from build123d import *

# Parameters (mm, degrees)
SKETCH1_R  = 1.25
BODY_DEPTH = 1.5


with BuildPart() as part:
    # Sketch1 → Body (new body)
    with BuildSketch(Plane.XY):
        with BuildLine():
            Line((6.047730211, -14.600512296), (7.232716872, -17.461323164))
            ThreePointArc((7.232716872, -17.461323164), (0, 18.9), (-7.232716872, -17.461323164))
            Line((-7.232716872, -17.461323164), (-6.047730211, -14.600512296))
            ThreePointArc((-6.047730211, -14.600512296), (-6.904744304, -11.609176709), (-10.012271945, -11.769905381))
            ThreePointArc((-10.012271945, -11.769905381), (-11.097089224, -12.142747822), (-12.128155002, -11.64001193))
            ThreePointArc((-12.128155002, -11.64001193), (0, 15.3), (12.128155002, -11.64001193))
            ThreePointArc((12.128155002, -11.64001193), (11.097089224, -12.142747822), (10.012271945, -11.769905381))
            ThreePointArc((10.012271945, -11.769905381), (6.904744304, -11.609176709), (6.047730211, -14.600512296))
        make_face()
        with Locations(Location((8.357429042, -13.643803715, 0), (0, 0, 180))):
            Circle(SKETCH1_R, mode=Mode.SUBTRACT)
        with Locations((-8.357429042, -13.643803715)):
            Circle(SKETCH1_R, mode=Mode.SUBTRACT)
    extrude(amount=-BODY_DEPTH)


solid = part.part
Model file for the job. Use its own axes, mm. A direction names the side the tool comes from. Round coordinates to 2 decimals unless told otherwise and drop trailing zeros. Loops run counter-clockwise (first coordinate to the right, second up) from the corner with the lowest first, then second, coordinate; pieces in that order, holes last. Notation, with made-up numbers: (-23, 24.5) - (-1, 24.5) arc R19 ccw to (-1, 38.5) - close; hole circle Ø4 at (29.5, 5.25). An arc over 180 degrees is marked (long way). Write each question's results on one line, items separated by ' | '.
(1) 3-axis set-ups, long thin cutter, end or side, ignore diameter. For faces 1 (the flat face through (0, 16, -1.5)), 2 (the cylindrical face through (-11.081, -12.144, -0.74)), 3 (the flat face through (6.63, -16.01, -0.74)): which of +Z, -Z, +X, -X, +Y, -Y reach the whole face in a straight line?
Answer below:
face 1: -Z, +X, -X, +Y, -Y | face 2: +Z, -Z | face 3: +Z, -Z, -Y
(2) Saw through at B-B, the plane x = 11. List the corners of the cut face in (y, z).
Answer below:
outline: (-15.37, -1.5) - (-12.15, -1.5) - (-12.15, 0) - (-15.37, 0) - close; (10.99, -1.5) - (15.37, -1.5) - (15.37, 0) - (10.99, 0) - close
(3) Saw through at D-D, the plane z = -1.1. List the corners of the cut face in (x, y).
Answer below:
outline: (-12.13, -11.64) arc R16.2 cw (long way) to (12.13, -11.64) arc R1.5 cw to (10.01, -11.77) arc R2.5 ccw to (6.05, -14.6) - (7.23, -17.46) arc R18.9 ccw (long way) to (-7.23, -17.46) - (-6.05, -14.6) arc R2.5 ccw to (-10.01, -11.77) arc R1.5 cw to start; hole circle Ø2.5 at (-8.36, -13.64); hole circle Ø2.5 at (8.36, -13.64)
(4) Saw through at C-C, the plane x = -8.5. List the corners of the cut face in (y, z), then the cut area to 3 significant figures.
Answer below:
outline: (-16.88, -1.5) - (-14.89, -1.5) - (-14.89, 0) - (-16.88, 0) - close; (-12.4, -1.5) - (-11.15, -1.5) - (-11.15, 0) - (-12.4, 0) - close; (12.89, -1.5) - (16.88, -1.5) - (16.88, 0) - (12.89, 0) - close | area: 10.9 mm^2
(5) Saw through at A-A, the plane y = 5. List the corners of the cut face in (x, z), then the cut area to 3 significant figures.
Answer below:
outline: (-18.23, -1.5) - (-15.09, -1.5) - (-15.09, 0) - (-18.23, 0) - close; (15.09, -1.5) - (18.23, -1.5) - (18.23, 0) - (15.09, 0) - close | area: 9.42 mm^2
(6) Wall check: L1, parallel to X at y = -13.5, z = -0.75; L2, parallel to Y at x = -9.5, z = -0.3; L3, parallel to Y at x = 0, z = -0.25. Give the ranges that are in metal, low to high.
Answer below:
L1: x = -13.23 to -9.6, -7.12 to -5.86, 5.86 to 7.12, 9.6 to 13.23 | L2: y = -16.34 to -14.15, -13.14 to -11.42, 12.22 to 16.34 | L3: y = 15.3 to 18.9
(7) Mould opens along X. For faces 4 (the cylindrical face through (0.727, 18.886, -0.74)), 5 (the cylindrical face through (-6.867, -11.637, -0.74)), 6 (the flat face through (0, 16, 0)) say: released by +X, released by -X, zero draft, split by the parting line, or undercut.
Answer below:
face 4: split by the parting line | face 5: undercut | face 6: zero draft
